Design review of the part built by this model. Coordinates are the model's own, in mm. A direction names the side the tool comes from. Coordinates: 2 decimals unless noted, no trailing zeros. Loops run counter-clockwise (first coordinate to the right, second up) from the corner with the lowest first, then second, coordinate; pieces in that order, holes last. Notation, with made-up numbers: M -38.75,-11.5 L -8.75,-11.5 A26 ccw -8.75,5.5 Z; hole C 46.5,3.25 d1. An arc over 180 degrees is marked long. One line per item, written item: value.
```python
from build123d import *

# Parameters (mm, degrees)
SKETCH1_W           = 40
SKETCH1_H           = 50
BOSS_EXTRUDE1_DEPTH = 10
BOSS_EXTRUDE2_DEPTH = 10
BOSS_EXTRUDE3_DEPTH = 40
BOSS_EXTRUDE4_DEPTH = 30
SKETCH5_R           = 8
CUT_EXTRUDE1_DEPTH  = 50
SKETCH6_R           = 16.35789331
SKETCH6_R_2         = 8
BOSS_EXTRUDE5_DEPTH = 10


with BuildPart() as part:
    # Sketch1 → Boss-Extrude1 (new body)
    with BuildSketch(Plane(origin=(0, 0, 0), x_dir=(1, 0, 0), z_dir=(0, 1, 0))):
        Rectangle(SKETCH1_W, SKETCH1_H)
    extrude(amount=BOSS_EXTRUDE1_DEPTH)

    # Sketch2 → Boss-Extrude2 (add)
    with BuildSketch(Plane(origin=(0, 10, 0), x_dir=(1, 0, 0), z_dir=(0, 1, 0))):
        Polygon((28, -15), (60, -15), (60, -5), (70, -5), (70, -25), (20, -25), (20, -15), (20, -7), align=None)
        Polygon((20, 25), (70, 25), (70, 5), (60, 5), (60, 15), (28, 15), (20, 7), (20, 15), align=None)
    extrude(amount=-BOSS_EXTRUDE2_DEPTH)

    # Sketch3 → Boss-Extrude3 (add)
    with BuildSketch(Plane.ZY.offset(20)):
        Polygon((-25, 10), (-35, 10), (-35, -50), (35, -50), (35, 10), (25, 10), (25, 0), (25, -40), (-25, -40), (-25, 0), align=None)
    extrude(amount=-BOSS_EXTRUDE3_DEPTH)

    # Sketch4 → Boss-Extrude4 (add)
    with BuildSketch(Plane(origin=(0, 10, 0), x_dir=(1, 0, 0), z_dir=(0, 1, 0))):
        Polygon((20, 7), (28, 15), (60, 15), (60, 5), (70, 5), (70, 25), (3.779860002, 25), (3.779860002, -25), (70, -25), (70, -5), (60, -5), (60, -15), (28, -15), (20, -7), align=None)
    extrude(amount=BOSS_EXTRUDE4_DEPTH)

    # Sketch5 → Cut-Extrude1 (cut)
    with BuildSketch(Plane(origin=(0, 0, -25), x_dir=(-1, 0, 0), z_dir=(0, 0, -1))):
        with Locations((-40, 22)):
            Circle(SKETCH5_R)
    extrude(amount=-CUT_EXTRUDE1_DEPTH, mode=Mode.SUBTRACT)

    # Sketch6 → Boss-Extrude5 (add)
    with BuildSketch(Plane.XY.offset(25)):
        with Locations(Location((40, 22, 0), (0, 0, 180))):
            Circle(SKETCH6_R)
        with Locations(Location((40, 22, 0), (0, 0, 180))):
            Circle(SKETCH6_R_2, mode=Mode.SUBTRACT)
    extrude(amount=BOSS_EXTRUDE5_DEPTH)


solid = part.part
```
(1) To check wall thickness, follow line 1 along Y through (x, z) = (-2, -0.5); line 2 along Z through (x, y) = (-11, -37.5); line 3 along Y through (x, z) = (18, -6). State the ranges of each line that lie inside material, in increasing order. Write a range as [from, to].
Reply:
line 1: y = [-50, -40], [0, 10]
line 2: z = [-35, -25], [25, 35]
line 3: y = [-50, -40], [0, 40]
(2) We need section D-D on y = -30.5. State the section outline as (x, z) points, then the cut area to 3 significant figures.
Reply:
outline: M -20,-35 L 20,-35 L 20,-25 L -20,-25 Z; M -20,25 L 20,25 L 20,35 L -20,35 Z
area: 800 mm2
(3) We need section C-C on x = 40. State the section outline as (y, z) points, then the cut area to 3 significant figures.
Reply:
outline: M 0,-25 L 14,-25 L 14,-15 L 0,-15 Z; M 0,15 L 14,15 L 14,35 L 5.64,35 L 5.64,25 L 0,25 Z; M 30,-25 L 40,-25 L 40,-15 L 30,-15 Z; M 30,15 L 40,15 L 40,25 L 38.36,25 L 38.36,35 L 30,35 Z
area: 647 mm2
(4) Tool access review of faces 1 (the flat face through (0, -40, 0)), 2 (the flat face through (65, 20, -5)), 3 (the flat face through (60, 20, -10)): name each direction out of +Z, -Z, +X, -X, +Y, -Y from which nothing blocks a thin tool from reaching the whole face with its end or side.
Reply:
face 1: +X, -X
face 2: +X, +Y, -Y
face 3: +Y, -Y
(5) We need section A-A on y = 22. State the section outline as (x, z) points, then the cut area to 3 significant figures.
Reply:
outline: M 3.78,-25 L 32,-25 L 32,-15 L 28,-15 L 20,-7 L 20,7 L 28,15 L 32,15 L 32,35 L 23.64,35 L 23.64,25 L 3.78,25 Z; M 48,-25 L 70,-25 L 70,-5 L 60,-5 L 60,-15 L 48,-15 Z; M 48,15 L 60,15 L 60,5 L 70,5 L 70,25 L 56.36,25 L 56.36,35 L 48,35 Z
area: 1,920 mm2
(6) We need section B-B on z = -12. State the section outline as (x, y) points, then the cut area to 3 significant figures.
Reply:
outline: M -20,-50 L 20,-50 L 20,-40 L -20,-40 Z; M -20,0 L 25,0 L 25,40 L 3.78,40 L 3.78,10 L -20,10 Z; M 60,0 L 70,0 L 70,40 L 60,40 Z
area: 1,890 mm2
(7) Mouldability with a two-part tool opening along X and no side actions: class faces 4 (the flat face through (24, 20, -11)), 5 (the flat face through (48, 20, 15)), 6 (the flat face through (-5, 10, 0)), 7 (the flat face through (-20, 0.4, -0.5)) as released by +X, released by -X, zero draft, split by the parting line, or undercut.
Reply:
face 4: undercut
face 5: undercut
face 6: zero draft
face 7: released by -X
(8) Insertion check: pin 1 (15.5 mm diameter, centred on y = 19.5, z = 1.5, fed in from +X); pin 2 (5 mm diameter, centred on y = 27.5, z = -12, fed in from -X); pin 3 (10 mm diameter, centred on y = -28.5, z = -25, fed in from +X); pin 4 (16 mm diameter, centred on x = 46.5, y = 22.5, fed in from -Z). Each pin has a flat end and moves straight along its axis. Give the tip position at first contact, or say it passes through.
Reply:
pin 1: stops at x = 70
pin 2: stops at x = 3.78
pin 3: stops at x = 20
pin 4: stops at z = -25
